Input: part model. Units: mm. Frame: model coordinates. A direction names the side the tool comes from. Give positions to 0.01 mm unless a question says otherwise; leave off trailing zeros. One line per item, written item: value. Start each with the question number.
(1) Pin query (flat end, axial travel): P1, Ø3.5, axis at x = -102, y = 2, coming from the +Z side. Return the tip coordinate at first contact, or that it passes through.
(2) Access query for faces 1 (the cylindrical face through (97, 0, 12)), 2 (the flat face through (-8, 0, 15)). Directions: +Z, -Z, +X, -X, +Y, -Y. A direction counts if a zero-diameter tool reaches every point of the face in a straight line with its end or side. Return the directions, or none.
(3) Section A-A on y = 0. State how many separate pieces and enclosed holes the cut face has, plus the area to 3 significant figures.
(4) Pull-direction query (X, two-part tool) for faces 3 (the flat face through (-8, 10, 7)), 4 (the flat face through (332.5, 0, 7)), 5 (the cylindrical face through (-108, 0, 12)); classes: released by +X, released by -X, zero draft, split by the parting line, or undercut.
(5) Ray query, line 1 along Y through (x, z) = (307.5, 13.5); line 2 along Y through (x, z) = (-102.5, 4); line 3 along X through (y, z) = (3, 3.25). Return the intervals inside material, ascending. Write a range as from..to.
```python
from build123d import *

# Parameters (mm, degrees)
SKETCH_1_W                = 665
SKETCH_1_H                = 20
EXTRUDE_1_DEPTH           = 15
HOLE_WIZARD_1_D           = 6.6
HOLE_WIZARD_1_CBORE_D     = 11
HOLE_WIZARD_1_CBORE_DEPTH = 6.8
SKETCH_5_W                = 15
SKETCH_5_H                = 20
EXTRUDE_2_DEPTH           = 25


with BuildPart() as part:
    # 草图1 → 凸台-拉伸1 (new body)
    with BuildSketch(Plane.XY):
        Rectangle(SKETCH_1_W, SKETCH_1_H)
    extrude(amount=EXTRUDE_1_DEPTH)

    # 打孔尺寸(%根据)内六角圆柱头螺钉的类型1 (through all)
    with Locations(Plane.XY.offset(15)):
        with Locations((102.5, 0), (-307.5, 0), (307.5, 0), (-102.5, 0)):
            CounterBoreHole(HOLE_WIZARD_1_D / 2, HOLE_WIZARD_1_CBORE_D / 2, HOLE_WIZARD_1_CBORE_DEPTH)

    # 草图5 → 凸台-拉伸2 (add)
    with BuildSketch(Plane.ZY.offset(332.5)):
        with Locations((7.5, 0)):
            Rectangle(SKETCH_5_W, SKETCH_5_H)
    extrude(amount=EXTRUDE_2_DEPTH)


solid = part.part
```
Output values:
1. P1: stops at z = 8.2
2. face 1: +Z
2. face 2: +Z, +X, -X, +Y, -Y
3. separate pieces: 5
3. enclosed holes: 0
3. area: 9,830 mm²
4. face 3: zero draft
4. face 4: released by +X
4. face 5: undercut
5. line 1: y = -10..-5.5, 5.5..10
5. line 2: y = -10..-3.3, 3.3..10
5. line 3: x = -357.5..-308.87, -306.13..-103.87, -101.13..101.13, 103.87..306.13, 308.87..332.5
